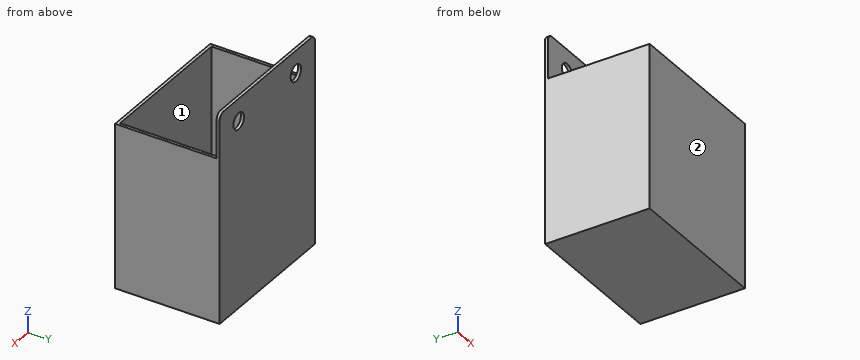
```python
from build123d import *

# Parameters (mm, degrees)
SKETCH_1_W          = 50
SKETCH_1_H          = 35
EXTRUDE_1_DEPTH     = 55
SKETCH_2_W          = 48
SKETCH_2_H          = 33
CUT_EXTRUDE_1_DEPTH = 54
SKETCH_5_W          = 50
SKETCH_5_H          = 1
EXTRUDE_2_DEPTH     = 15
SKETCH_6_R          = 2.75
CUT_EXTRUDE_3_DEPTH = 12
FILLET_1_R          = 2


with BuildPart() as part:
    # 草图1 → 凸台-拉伸1 (new body)
    with BuildSketch(Plane.XY):
        Rectangle(SKETCH_1_W, SKETCH_1_H)
    extrude(amount=EXTRUDE_1_DEPTH)

    # 草图2 → 切除-拉伸1 (cut)
    with BuildSketch(Plane.XY.offset(55)):
        Rectangle(SKETCH_2_W, SKETCH_2_H)
    extrude(amount=-CUT_EXTRUDE_1_DEPTH, mode=Mode.SUBTRACT)

    # 草图5 → 凸台-拉伸2 (add)
    with BuildSketch(Plane.XY.offset(55)):
        with Locations((0, 17)):
            Rectangle(SKETCH_5_W, SKETCH_5_H)
    extrude(amount=EXTRUDE_2_DEPTH)

    # 草图6 → 切除-拉伸3 (cut)
    with BuildSketch(Plane.XZ.offset(-16.5)):
        with Locations(Location((-15, 62.5, 0), (0, 0, 270))):
            Circle(SKETCH_6_R)
        with Locations(Location((15, 62.5, 0), (0, 0, 270))):
            Circle(SKETCH_6_R)
    extrude(amount=-CUT_EXTRUDE_3_DEPTH, mode=Mode.SUBTRACT)

    # 圆角1
    fillet_1_edges = [part.edges().sort_by_distance(p)[0] for p in [
        (25, 17, 70),
        (-25, 17, 70),
    ]]
    fillet(fillet_1_edges, radius=FILLET_1_R)


solid = part.part
```
Could you check a few things on this model? Use its own coordinates, in mm. Face numbers are marked on the shaded views. A direction names the side the tool comes from. Coordinates: 2 decimals unless noted, no trailing zeros. Order: outer loops, then holes, each group sorted by start corner. A loop starts at its lowest first (then second) coordinate and runs counter-clockwise, first axis right, second up. Notation, with made-up numbers: M 3,74.25 L 20,74.25 A19 cw 20,96.25 Z; hole C 19,-30 d6. An arc over 180 degrees is marked long. Use a Markdown table: item, result. Add a question column.
Q1. Which directions (+Z, -Z, +X, -X, +Y, -Y) give clear straight access to the entire face, cutting with the end or side of a thin tool? Please do the marked faces 1 and 2.
Q2. If I drill on L1, parallel to X at y = 16.75, z = 62.5; L2, parallel to X at y = -1, z = 53; L3, parallel to Y at x = 21.5, z = 23, over which ranges is the centre line in solid material (lowest first)?
Q3. I'm going to push flat-ended pins straight in: pin 1 (10 mm diameter, centred on x = 2.5, y = -5.5, fed in from +Z); pin 2 (3 mm diameter, centred on x = -0.5, y = -10, fed in from -Z); pin 3 (4.5 mm diameter, centred on x = -15, z = 62.5, fed in from +Y). Where does each tip first touch, or does it pass through?
Q4. I want a section at C-C on y = 11.5. List the corners of the cut face in (x, z) for me, then the cut area to 3 significant figures.
Q5. I want a section at B-B on z = 62.5. List the corners of the cut face in (x, y) for me.
Q6. I want a section at A-A on x = -15. List the corners of the cut face in (y, z) for me.
Q7. I want a section at D-D on x = -1. List the corners of the cut face in (y, z) for me, then the cut area to 3 significant figures.
Checked values:
| question | item | result |
|---|---|---|
| 1 | face 1 | +Z |
| 1 | face 2 | +Z, -Z, +X, -X, -Y |
| 2 | L1 | -25 to -17.75, -12.25 to 12.25, 17.75 to 25 |
| 2 | L2 | -25 to -24, 24 to 25 |
| 2 | L3 | -17.5 to -16.5, 16.5 to 17.5 |
| 3 | pin 1 | z = 1 |
| 3 | pin 2 | z = 0 |
| 3 | pin 3 | through |
| 4 | outline | M -25,0 L 25,0 L 25,55 L 24,55 L 24,1 L -24,1 L -24,55 L -25,55 Z |
| 4 | area | 158 mm² |
| 5 | outline | M -25,16.5 L -17.75,16.5 L -17.75,17.5 L -25,17.5 Z; M -12.25,16.5 L 12.25,16.5 L 12.25,17.5 L -12.25,17.5 Z; M 17.75,16.5 L 25,16.5 L 25,17.5 L 17.75,17.5 Z |
| 6 | outline | M -17.5,0 L 17.5,0 L 17.5,59.75 L 16.5,59.75 L 16.5,1 L -16.5,1 L -16.5,55 L -17.5,55 Z; M 16.5,65.25 L 17.5,65.25 L 17.5,70 L 16.5,70 Z |
| 7 | outline | M -17.5,0 L 17.5,0 L 17.5,70 L 16.5,70 L 16.5,1 L -16.5,1 L -16.5,55 L -17.5,55 Z |
| 7 | area | 158 mm² |
